from build123d import *

# Parameters (mm, degrees)
SKETCH_1_W              = 55
SKETCH_1_H              = 80
EXTRUDE_1_DEPTH         = 12
CUT_EXTRUDE_4_REACH     = 52.002
SKETCH_5_R              = 10
CHAMFER_1_SIZE          = 5
HOLE_WIZARD_M4_1_REACH  = 85.845
HOLE_WIZARD_M4_1_BORE_R = 1.65


with BuildPart() as part:
    # 草图1 → 凸台-拉伸1 (new body)
    with BuildSketch(Plane.XY):
        Rectangle(SKETCH_1_W, SKETCH_1_H)
    extrude(amount=EXTRUDE_1_DEPTH)

    # 草图5 → 切除-拉伸4 (cut, up to next)
    with BuildSketch(Plane(origin=(0, 0, 0), x_dir=(-1, 0, 0), z_dir=(0, 0, -1)), mode=Mode.PRIVATE) as cut_extrude_4_sk1:
        with Locations((0, 25)):
            Circle(SKETCH_5_R)
    cut_extrude_4_tool1 = extrude(cut_extrude_4_sk1.sketch, amount=-CUT_EXTRUDE_4_REACH, mode=Mode.PRIVATE) & part.part
    add(cut_extrude_4_tool1.solids().sort_by_distance((0, 25, 0))[0], mode=Mode.SUBTRACT)

    # 倒角1
    chamfer_1_edges = [part.edges().sort_by_distance(p)[0] for p in [
        (-27.5, 40, 6),
        (27.5, 40, 6),
    ]]
    chamfer(chamfer_1_edges, length=CHAMFER_1_SIZE)

    # M4 螺纹孔1 bore (on position points) → M4 螺纹孔1 (cut, up to next)
    with BuildSketch(Plane(origin=(27.5, 23, 6), x_dir=(0, 0, 1), z_dir=(1, 0, 0)), mode=Mode.PRIVATE) as hole_wizard_m4_1_sk1:
        Circle(HOLE_WIZARD_M4_1_BORE_R)
    hole_wizard_m4_1_tool1 = extrude(hole_wizard_m4_1_sk1.sketch, amount=-HOLE_WIZARD_M4_1_REACH, mode=Mode.PRIVATE) & part.part
    add(hole_wizard_m4_1_tool1.solids().sort_by_distance((27.5, 23, 6))[0], mode=Mode.SUBTRACT)


solid = part.part
Work out the finished part from the listing and answer in its coordinate system (mm). A direction names the side the tool comes from. Round coordinates to 2 decimals unless told otherwise and drop trailing zeros. Loops run counter-clockwise (first coordinate to the right, second up) from the corner with the lowest first, then second, coordinate; pieces in that order, holes last. Notation, with made-up numbers: M 52.5,69 L 90.5,69 A27 cw 90.5,97 Z; hole C -10,33.25 d8. An arc over 180 degrees is marked long. One line per question, with ' | ' between items. Start each with the question number.
(1) A tool of negligible diameter and unlimited length cuts with its end or side. For faces 1 (the face through (25, 37.5, 5.9)), 2 (the face through (18.532, 21.885, 4.784)), from which of +Z, -Z, +X, -X, +Y, -Y can it reach the whole face along a straight path? Write none if from no direction.
(2) Find the intervals of material crossed by line 1 (Z direction, x = 17.75, y = 23); line 2 (Y direction, x = 0, z = 6.5); line 3 (Y direction, x = 17, z = 6), in increasing order.
(3) A cutting plane is placed at A-A on x = 0. Write down the section's boundary in (y, z), plus the area to 3 significant figures.
(4) A cutting plane is placed at B-B on y = 27. Write down the section's boundary in (x, z), plus the area to 3 significant figures.
(5) A flat-ended cylindrical pin translates along its axis: pin 1 Ø1 at (x, y) = (-21.5, -9) entering from -Z. Find the tip coordinate at first contact, or state that the pin passes through.
(6) A cutting plane is placed at D-D on z = 5.25. Write down the section's boundary in (x, y), plus the area to 3 significant figures.
(7) For a pull along Y with two mould halves and no side action, classify faces 3 (the face through (1.302, 34.915, 5.916)), 4 (the face through (0, -40, 6)), 5 (the face through (0, 40, 6)) as released by +Y, released by -Y, zero draft, split by the parting line, or undercut.
(8) A cutting plane is placed at C-C on z = 8.75. Write down the section's boundary in (x, y).
Geometry check:
1) face 1: +Z, -Z, +X, +Y | face 2: +X
2) line 1: z = 0 to 4.35, 7.65 to 12 | line 2: y = -40 to 15, 35 to 40 | line 3: y = -40 to 21.35, 24.65 to 40
3) outline: M -40,0 L 15,0 L 15,12 L -40,12 Z; M 35,0 L 40,0 L 40,12 L 35,12 Z | area: 720 mm²
4) outline: M -27.5,0 L -9.8,0 L -9.8,12 L -27.5,12 Z; M 9.8,0 L 27.5,0 L 27.5,12 L 9.8,12 Z | area: 425 mm²
5) pin 1: stops at z = 0
6) outline: M -27.5,-40 L 27.5,-40 L 27.5,21.53 L 9.38,21.53 A10 cw long 9.99,24.47 L 27.5,24.47 L 27.5,35 L 22.5,40 L -22.5,40 L -27.5,35 Z | area: 4,010 mm²
7) face 3: undercut | face 4: released by -Y | face 5: released by +Y
8) outline: M -27.5,-40 L 27.5,-40 L 27.5,35 L 22.5,40 L -22.5,40 L -27.5,35 Z; hole C 0,25 d20
